Could you check a few things on this model? Use its own coordinates, in mm. Give positions to 0.01 mm unless a question says otherwise; leave off trailing zeros. Write each loop counter-clockwise with the first axis right and the second up, starting at its lowest first coordinate (ties: lowest second). Pieces come first, ordered by that corner, then holes. Notation, with made-up numbers: (60.25, 65) - (115.25, 65) arc R21 cw to (115.25, 73) - close; hole circle Ø11 at (1.5, -11.5). An arc over 180 degrees is marked (long way). Write item = value, one per line.
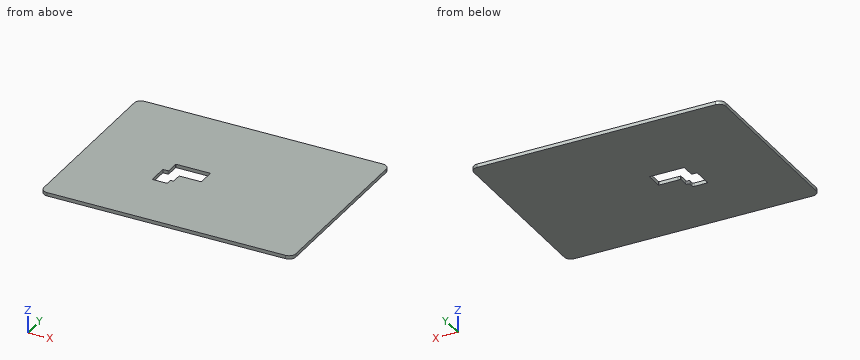
from build123d import *

# Parameters (mm, degrees)
EXTRUDE_1_DEPTH     = 15
CUT_EXTRUDE_1_DEPTH = 829.113419972


with BuildPart() as part:
    # 草图1 → 凸台-拉伸1 (new body)
    with BuildSketch(Plane.XY):
        with BuildLine():
            Line((-456.754393923, 478.74061611), (-456.754393923, -271.25938389))
            ThreePointArc((-456.754393923, -271.25938389), (-447.967597359, -292.472587326), (-426.754393923, -301.25938389))
            Line((-426.754393923, -301.25938389), (623.245606077, -301.25938389))
            ThreePointArc((623.245606077, -301.25938389), (644.458809512, -292.472587326), (653.245606077, -271.25938389))
            Line((653.245606077, -271.25938389), (653.245606077, 478.74061611))
            ThreePointArc((653.245606077, 478.74061611), (644.458809512, 499.953819545), (623.245606077, 508.74061611))
            Line((623.245606077, 508.74061611), (-426.754393923, 508.74061611))
            ThreePointArc((-426.754393923, 508.74061611), (-447.967597359, 499.953819545), (-456.754393923, 478.74061611))
        make_face()
    extrude(amount=EXTRUDE_1_DEPTH)

    # 草图2 → 切除-拉伸1 (cut, through all)
    with BuildSketch(Plane.XY.offset(15)):
        with BuildLine():
            Line((-113.754393923, 51.678144789), (-113.754393923, -13.321855211))
            ThreePointArc((-113.754393923, -13.321855211), (-112.289927829, -16.857389117), (-108.754393923, -18.321855211))
            Line((-108.754393923, -18.321855211), (-52.754393923, -18.321855211))
            ThreePointArc((-52.754393923, -18.321855211), (-49.218860017, -16.857389117), (-47.754393923, -13.321855211))
            Line((-47.754393923, -13.321855211), (-47.754393923, 3.746846437))
            ThreePointArc((-47.754393923, 3.746846437), (-46.31430038, 7.257838606), (-42.823567517, 8.746367915))
            Line((-42.823567517, 8.746367915), (-38.68522033, 8.803626264))
            ThreePointArc((-38.68522033, 8.803626264), (-35.194487466, 10.292155573), (-33.754393923, 13.803147743))
            Line((-33.754393923, 13.803147743), (-33.754393923, 51.678144789))
            Line((-33.754393923, 51.678144789), (-33.754393923, 53.24152579))
            ThreePointArc((-33.754393923, 53.24152579), (-33.016130918, 54.337823849), (-31.755279488, 54.734252116))
            Line((-31.755279488, 54.734252116), (-20.864600558, 54.67610792))
            Line((-20.864600558, 54.67610792), (62.197064842, 54.67610792))
            ThreePointArc((62.197064842, 54.67610792), (63.611278404, 55.261894358), (64.197064842, 56.67610792))
            Line((64.197064842, 56.67610792), (64.197064842, 89.975586232))
            Line((64.197064842, 89.975586232), (64.197064842, 128.216032673))
            ThreePointArc((64.197064842, 128.216032673), (63.611278404, 129.630246236), (62.197064842, 130.216032673))
            Line((62.197064842, 130.216032673), (-86.692151935, 130.216032673))
            ThreePointArc((-86.692151935, 130.216032673), (-88.106365497, 129.630246236), (-88.692151935, 128.216032673))
            Line((-88.692151935, 128.216032673), (-88.692151935, 100.216032673))
            Line((-88.692151935, 100.216032673), (-88.692151935, 72.429613021))
            ThreePointArc((-88.692151935, 72.429613021), (-89.277938372, 71.015399459), (-90.692151935, 70.429613021))
            Line((-90.692151935, 70.429613021), (-111.754393923, 70.429613021))
            ThreePointArc((-111.754393923, 70.429613021), (-113.168607486, 69.843826583), (-113.754393923, 68.429613021))
            Line((-113.754393923, 68.429613021), (-113.754393923, 51.678144789))
        make_face()
    extrude(amount=-CUT_EXTRUDE_1_DEPTH, mode=Mode.SUBTRACT)


solid = part.part
1. If we section it at B-B, the plane x = 28: Please give me the cut outline in (y, z).
Filled sheet:
outline = (-301.26, 0) - (54.68, 0) - (54.68, 15) - (-301.26, 15) - close; (130.22, 0) - (508.74, 0) - (508.74, 15) - (130.22, 15) - close
2. I need wall thicknesses on line 1 (Y direction, x = -67, z = 10.75); line 2 (X direction, y = 67.5, z = 10.25); line 3 (X direction, y = 119, z = 12.25). Which ranges of each line are inside material? Lowest first, please.
Filled sheet:
line_1 = -301.26 to -18.32, 130.22 to 508.74
line_2 = -456.75 to -113.75, 64.2 to 653.25
line_3 = -456.75 to -88.69, 64.2 to 653.25
3. If we section it at A-A, the plane y = 34.5: Please give me the cut outline in (x, z), and give its area (4 significant figures).
Filled sheet:
outline = (-456.75, 0) - (-113.75, 0) - (-113.75, 15) - (-456.75, 15) - close; (-33.75, 0) - (653.25, 0) - (653.25, 15) - (-33.75, 15) - close
area = 15,450 mm2
